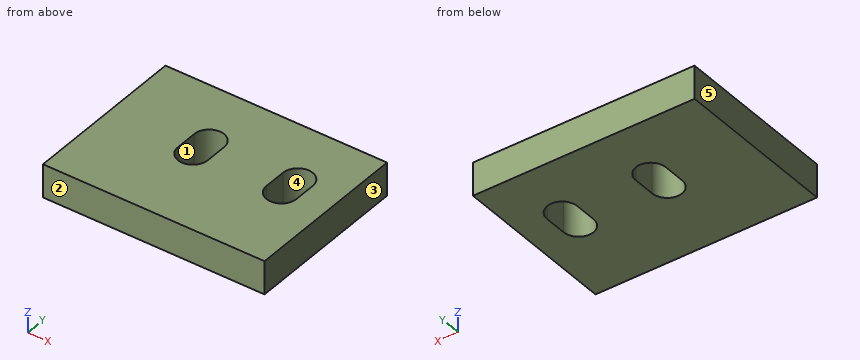
```python
from build123d import *

# Parameters (mm, degrees)
SKETCH1_W           = 200
SKETCH1_H           = 150
BOSS_EXTRUDE1_DEPTH = 30


with BuildPart() as part:
    # Sketch1 → Boss-Extrude1 (new body)
    with BuildSketch(Plane.XY):
        with Locations((100, 75)):
            Rectangle(SKETCH1_W, SKETCH1_H)
        with BuildLine():
            Line((93.5, 95), (93.5, 75))
            ThreePointArc((93.5, 75), (80, 61.5), (66.5, 75))
            Line((66.5, 75), (66.5, 95))
            ThreePointArc((66.5, 95), (80, 108.5), (93.5, 95))
        make_face(mode=Mode.SUBTRACT)
        with BuildLine():
            Line((173.5, 95), (173.5, 75))
            ThreePointArc((173.5, 75), (160, 61.5), (146.5, 75))
            Line((146.5, 75), (146.5, 95))
            ThreePointArc((146.5, 95), (160, 108.5), (173.5, 95))
        make_face(mode=Mode.SUBTRACT)
    extrude(amount=BOSS_EXTRUDE1_DEPTH)


solid = part.part
```
Input: part model. Units: mm. Frame: model coordinates. Face numbers are marked on the shaded views. A direction names the side the tool comes from. Coordinates: 2 decimals unless noted, no trailing zeros. Loops run counter-clockwise (first coordinate to the right, second up) from the corner with the lowest first, then second, coordinate; pieces in that order, holes last. Notation, with made-up numbers: M 24.25,66.25 L 82.25,66.25 A21 cw 82.25,88.25 Z; hole C 24,24 d3. An arc over 180 degrees is marked long. Answer in a Markdown table with one row per item.
1. Reachability of the marked faces 4 and 5 from +Z, -Z, +X, -X, +Y, -Y: full face, straight path, thin tool, end or side. Return the list, or none.
Response:
| item | result |
|---|---|
| face 4 | +Z, -Z |
| face 5 | +Z, -Z, -X, +Y, -Y |
2. Section A-A, the plane x = 80. Output: boundary loops of the cut face in (y, z), then the cut area to 3 significant figures.
Response:
| item | result |
|---|---|
| outline | M 0,0 L 61.5,0 L 61.5,30 L 0,30 Z; M 108.5,0 L 150,0 L 150,30 L 108.5,30 Z |
| area | 3,090 mm2 |
3. Draft query along Y for the marked faces 1, 2 and 3. Return one class per face: pulls with the +Y half, pulls with the -Y half, needs draft (parallel to the pull), parting line crosses it, or undercut.
Response:
| item | result |
|---|---|
| face 1 | undercut |
| face 2 | pulls with the -Y half |
| face 3 | needs draft |
4. Section C-C, the plane y = 98.5. Output: boundary loops of the cut face in (x, z).
Response:
| item | result |
|---|---|
| outline | M 0,0 L 66.96,0 L 66.96,30 L 0,30 Z; M 93.04,0 L 146.96,0 L 146.96,30 L 93.04,30 Z; M 173.04,0 L 200,0 L 200,30 L 173.04,30 Z |
5. Section B-B, the plane z = 12.75. Output: boundary loops of the cut face in (x, y), then the cut area to 3 significant figures.
Response:
| item | result |
|---|---|
| outline | M 0,0 L 200,0 L 200,150 L 0,150 Z; hole M 66.5,75 A13.5 ccw 93.5,75 L 93.5,95 A13.5 ccw 66.5,95 Z; hole M 146.5,75 A13.5 ccw 173.5,75 L 173.5,95 A13.5 ccw 146.5,95 Z |
| area | 27,800 mm2 |
6. Material intervals for line 1 (X direction, y = 79, z = 19); line 2 (X direction, y = 104, z = 23); line 3 (Y direction, x = 72, z = 22.25), sorted ascending.
Response:
| item | result |
|---|---|
| line 1 | x = 0 to 66.5, 93.5 to 146.5, 173.5 to 200 |
| line 2 | x = 0 to 69.94, 90.06 to 149.94, 170.06 to 200 |
| line 3 | y = 0 to 64.13, 105.87 to 150 |
